Build history of the part. All positions in model axes, mm. A direction names the side the tool comes from. Round coordinates to 2 decimals unless told otherwise and drop trailing zeros. Write each loop counter-clockwise with the first axis right and the second up, starting at its lowest first coordinate (ties: lowest second). Pieces come first, ordered by that corner, then holes. Notation, with made-up numbers: M -24,77 L 31,77 A18 cw 31,102 Z; hole C -27,21 d7. An arc over 180 degrees is marked long. Write item = value, one per line. Start each with the question number.
Q1. Band-saw the part on C-C on x = 39. Write the cut outline in (y, z).
Q2. Probe L1, parallel to X at y = -20, z = -35; L2, parallel to Z at x = 7.5, y = 23.5; L3, parallel to X at y = 29, z = 25. List the from-to ranges inside material, lowest first.
Q3. Tool access for faces 4 (the cylindrical face through (39.692, 0.66, 14.985)), 5 (the flat face through (0, 1, 1)), 6 (the cylindrical face through (7.395, -25.724, -29.142)), 7 (the cylindrical face through (72.395, -20.628, 17.049)): list every direction of +Z, -Z, +X, -X, +Y, -Y with a clear straight run to the whole face (end or side of a thin tool).
Q4. Band-saw the part on A-A on y = 0. Write the cut outline in (x, z).
Q5. Band-saw the part on D-D on z = -16.5. State how many separate pieces and enclosed holes the cut face has, plus the area to 3 significant figures.
Q6. Drop flat-ended pins along their axis: P1, Ø2, axis at x = 65, y = 9, coming from the +Z side; P2, Ø8, axis at x = 36, y = 7, coming from the +Z side; P3, Ø4, axis at y = -17.7, z = -17.7, coming from the +X side. Give the stop position or say it passes through.
Q7. Pull direction Y, two halves, no side cores. Call faces 1 (the flat face through (80, 1, 1)), 2 (the cylindrical face through (7.395, -29.142, 25.724)), 3 (the cylindrical face through (72.42, 15.02, -47.69)): released by +Y, released by -Y, zero draft, split by the parting line, or undercut.
```python
from build123d import *

# Parameters (mm, degrees)
SKETCH_1_R                = 50
EXTRUDE_1_DEPTH           = 15
SKETCH_2_R                = 15
EXTRUDE_2_DEPTH           = 50
SKETCH_3_R                = 50
EXTRUDE_3_DEPTH           = 15
HOLE_WIZARD_7_0_7_1_D     = 7
HOLE_WIZARD_7_0_7_1_DEPTH = 19.75
HOLE_WIZARD_7_0_7_1_TIP   = 2.103012167
MM_1_D                    = 6
MM_1_DEPTH                = 19.75
MM_1_TIP                  = 1.802581857
PATTERN_CIRCULAR_1_COUNT  = 4
FILLET_1_R                = 3
CHAMFER_1_SIZE            = 2


with BuildPart() as part:
    # 草图1 → 凸台-拉伸1 (new body)
    with BuildSketch(Plane(origin=(0, 0, 0), x_dir=(0, 0, -1), z_dir=(1, 0, 0))):
        Circle(SKETCH_1_R)
    extrude(amount=EXTRUDE_1_DEPTH)

    # 草图2 → 凸台-拉伸2 (add)
    with BuildSketch(Plane(origin=(15, 0, 0), x_dir=(0, 0, -1), z_dir=(1, 0, 0))):
        Circle(SKETCH_2_R)
    extrude(amount=EXTRUDE_2_DEPTH)

    # 草图3 → 凸台-拉伸3 (add)
    with BuildSketch(Plane(origin=(65, 0, 0), x_dir=(0, 0, -1), z_dir=(1, 0, 0))):
        Circle(SKETCH_3_R)
    extrude(amount=EXTRUDE_3_DEPTH)

    # Ø7.0 (7) 直径孔1
    with Locations(Plane(origin=(80, 0, 0), x_dir=(0, 0, -1), z_dir=(1, 0, 0))):
        with Locations((-17.698882733, 17.698882733), (17.698882733, -17.698882733)):
            Hole(HOLE_WIZARD_7_0_7_1_D / 2, depth=HOLE_WIZARD_7_0_7_1_DEPTH)
            with Locations((0, 0, -(HOLE_WIZARD_7_0_7_1_DEPTH + HOLE_WIZARD_7_0_7_1_TIP / 2))):  # 118° drill point
                Cone(0, HOLE_WIZARD_7_0_7_1_D / 2, HOLE_WIZARD_7_0_7_1_TIP, mode=Mode.SUBTRACT)

    # 大小mm 暗销孔1
    with Locations(Plane(origin=(80, 0, 0), x_dir=(0, 0, -1), z_dir=(1, 0, 0))):
        with Locations((-17.698882733, -17.698882733), (17.698882733, 17.698882733)):
            Hole(MM_1_D / 2, depth=MM_1_DEPTH)
            with Locations((0, 0, -(MM_1_DEPTH + MM_1_TIP / 2))):  # 118° drill point
                Cone(0, MM_1_D / 2, MM_1_TIP, mode=Mode.SUBTRACT)

    # 草图9 → Ø9.0 (9) 直径孔1 (revolve, cut)
    with BuildSketch(Plane(origin=(0, 24.748737342, -24.748737342), x_dir=(0, 0, 1), z_dir=(0, 1, 0))):
        Polygon((0, 0), (0, 22.453872786), (4.5, 19.75), (4.5, 0), align=None)
    hole_wizard_9_0_9_1 = revolve(axis=Axis((-6.35, 24.748737342, -24.748737342), (1, 0, 0)), mode=Mode.SUBTRACT)

    # 阵列(圆周)1: Ø9.0 (9) 直径孔1 ×4 about axis
    pattern_circular_1_axis = Axis((0, 0, 0), (1, 0, 0))
    for i in range(1, PATTERN_CIRCULAR_1_COUNT):
        add(hole_wizard_9_0_9_1.rotate(pattern_circular_1_axis, i * 360 / PATTERN_CIRCULAR_1_COUNT), mode=Mode.SUBTRACT)

    # 圆角1
    fillet_1_edges = [part.edges().sort_by_distance(p)[0] for p in [
        (15, 0, 15),
        (65, 0, 15),
    ]]
    fillet(fillet_1_edges, radius=FILLET_1_R)

    # 倒角1
    chamfer_1_edges = [part.edges().sort_by_distance(p)[0] for p in [
        (0, 0, 50),
        (15, 0, 50),
        (65, 0, 50),
        (80, 0, 50),
    ]]
    chamfer(chamfer_1_edges, length=CHAMFER_1_SIZE)


solid = part.part
```
Conclusion:
q1.outline = C 0,0 d30
q2.L1 = 0 to 15, 65 to 80
q2.L2 = -44.13 to -29.07, -20.43 to 20.43, 29.07 to 44.13
q2.L3 = 65 to 80
q3.face_4 = none
q3.face_5 = +Z, -Z, -X, +Y, -Y
q3.face_6 = -X
q3.face_7 = +X
q4.outline = M 0,-48 L 2,-50 L 13,-50 L 15,-48 L 15,-18 A3 cw 18,-15 L 62,-15 A3 cw 65,-18 L 65,-48 L 67,-50 L 78,-50 L 80,-48 L 80,48 L 78,50 L 67,50 L 65,48 L 65,18 A3 cw 62,15 L 18,15 A3 cw 15,18 L 15,48 L 13,50 L 2,50 L 0,48 Z
q5.separate_pieces = 4
q5.enclosed_holes = 0
q5.area = 2,640 mm^2
q6.P1 = 48.18
q6.P2 = 14.7
q6.P3 = 15
q7.face_1 = zero draft
q7.face_2 = undercut
q7.face_3 = split by the parting line
